Check sheet for the modelled part. Datum: model origin and axes. Units: mm. A direction names the side the tool comes from. Give positions to 0.01 mm unless a question says otherwise; leave off trailing zeros. Order: outer loops, then holes, each group sorted by start corner. A loop starts at its lowest first (then second) coordinate and runs counter-clockwise, first axis right, second up. Notation, with made-up numbers: (18.25, 75) -> (63.25, 75) arc R28 cw to (63.25, 111) -> close; hole circle Ø11 at (42, 76.5). An arc over 180 degrees is marked (long way). Answer in a Markdown table with one row per item. Add a question column.
(1) Go/stop test with flat-tipped pins: pin 1 (24.5 mm diameter, centred on y = -59.5, z = -32, fed in from -X); pin 2 (7 mm diameter, centred on x = -9, z = -56.5, fed in from -Y); pin 3 (12 mm diameter, centred on y = -108.5, z = -31.5, fed in from +X) (3 decimals); pin 4 (5 mm diameter, centred on y = -75.5, z = -14, fed in from -X) (3 decimals). Record where each tip stops, or that it passes through.
(2) Cross-section at A-A (x = 3). Record the cut outline in (y, z) (3 decimals).
(3) Release check for a two-part mould opening along Z. For faces 3 (the face through (10.414, -42, -28)), 4 (the face through (17.145, -96.1, -52.3)), 5 (the face through (-0.263, -75.988, -39.746)) record: released by +Z, released by -Z, zero draft, split by the parting line, or undercut.
(4) Thickness scan on L1, parallel to Z at x = -10, y = -76; L2, parallel to Y at x = 12, z = -20; L3, parallel to Y at x = -11.5, z = -29. Record the ranges inside material, lowest first. Write a range as [from, to].
(5) Set-up check for faces 1 (the face through (-10.414, -42, -28)), 2 (the face through (14.12, -61.63, -33.01)): record each of +Z, -Z, +X, -X, +Y, -Y from which the full face is reachable in a straight line by a thin tool's end or side.
```python
from build123d import *

# Parameters (mm, degrees)
BOSS_EXTRUDE1_DEPTH      = 17.145
BOSS_EXTRUDE1_DEPTH_BACK = 17.145
SKETCH1_R                = 62.865
SKETCH2_R                = 46.355
SKETCH2_R_2              = 33.655
CUT_EXTRUDE1_DEPTH       = 6.731
SKETCH3_R                = 26.289
CUT_EXTRUDE2_DEPTH       = 10.16
BOSS_EXTRUDE2_DEPTH      = 18.796
BOSS_EXTRUDE2_DEPTH_BACK = 18.796
SKETCH4_R                = 14.2875
FILLET1_R                = 6.35
DRAFT1_ANGLE             = 5
DRAFT2_ANGLE             = 5
SKETCH5_R                = 4.826
CUT_EXTRUDE3_DEPTH       = 175.112368419
SKETCH6_W                = 11.857056217
SKETCH6_H                = 6.35
EXTRUDE_THIN1_DEPTH      = 6.35


with BuildPart() as part:
    # Sketch1 → Boss-Extrude1 (new, two sides: drawn at the far end of the back side and taken through both)
    with BuildSketch(Plane(origin=(0, 0, 0), x_dir=(0, 0, -1), z_dir=(1, 0, 0)).offset(-BOSS_EXTRUDE1_DEPTH_BACK)):
        with Locations((34.925, -76.2)):
            Circle(SKETCH1_R)
    extrude(amount=BOSS_EXTRUDE1_DEPTH + BOSS_EXTRUDE1_DEPTH_BACK)

    # Sketch2 → Cut-Extrude1 (cut)
    with BuildSketch(Plane.ZY.offset(17.145)):
        with Locations((-34.925, -76.2)):
            Circle(SKETCH2_R)
        with Locations((-34.925, -76.2)):
            Circle(SKETCH2_R_2, mode=Mode.SUBTRACT)
    cut_extrude1 = extrude(amount=-CUT_EXTRUDE1_DEPTH, mode=Mode.SUBTRACT)

    # Sketch3 → Cut-Extrude2 (cut)
    with BuildSketch(Plane.ZY.offset(17.145)):
        with Locations((-34.925, -76.2)):
            Circle(SKETCH3_R)
    cut_extrude2 = extrude(amount=-CUT_EXTRUDE2_DEPTH, mode=Mode.SUBTRACT)

    # Mirror1: Cut-Extrude1, Cut-Extrude2 across plane
    add(cut_extrude1.mirror(Plane(origin=(0, 0, 0), x_dir=(0, 0, 1), z_dir=(1, 0, 0))), mode=Mode.SUBTRACT)
    add(cut_extrude2.mirror(Plane(origin=(0, 0, 0), x_dir=(0, 0, 1), z_dir=(1, 0, 0))), mode=Mode.SUBTRACT)

    # Sketch4 → Boss-Extrude2 (add, two sides: drawn at the far end of the back side and taken through both)
    with BuildSketch(Plane(origin=(0, 0, 0), x_dir=(0, 0, -1), z_dir=(1, 0, 0)).offset(-BOSS_EXTRUDE2_DEPTH_BACK)):
        with Locations((34.925, -76.2)):
            Circle(SKETCH4_R)
    extrude(amount=BOSS_EXTRUDE2_DEPTH + BOSS_EXTRUDE2_DEPTH_BACK)

    # Fillet1
    fillet1_edges = [part.edges().sort_by_distance(p)[0] for p in [
        (-17.145, -76.2, 27.94),
        (17.145, -76.2, 27.94),
    ]]
    fillet(fillet1_edges, radius=FILLET1_R)

    # Draft1
    draft1_faces = [part.faces().sort_by_distance(p)[0] for p in [
        (-13.7795, -76.2, -81.28),
        (-13.7795, -76.2, -68.58),
        (-12.065, -76.2, -61.214),
        (-12.8905, -76.2, -20.6375),
    ]]
    draft(draft1_faces, Plane(origin=(-18.796, -76.2, -34.925), x_dir=(0, 0, -1), z_dir=(-1, 0, 0)), DRAFT1_ANGLE)

    # Draft2
    draft2_faces = [part.faces().sort_by_distance(p)[0] for p in [
        (13.7795, -76.2, -81.28),
        (13.7795, -76.2, -68.58),
        (12.065, -76.2, -61.214),
        (12.8905, -76.2, -20.6375),
    ]]
    draft(draft2_faces, Plane(origin=(18.796, -76.2, -34.925), x_dir=(0, 0, 1), z_dir=(1, 0, 0)), DRAFT2_ANGLE)

    # Sketch5 → Cut-Extrude3 (cut, through all)
    with BuildSketch(Plane.ZY.offset(18.796)):
        with Locations((-34.925, -76.2)):
            Circle(SKETCH5_R)
    extrude(amount=-CUT_EXTRUDE3_DEPTH, mode=Mode.SUBTRACT)

    # Sketch6 → Extrude-Thin1 (add)
    with BuildSketch(Plane.ZY.offset(6.985)):
        with Locations((-55.141028109, -76.2)):
            Rectangle(SKETCH6_W, SKETCH6_H)
        with Locations((-14.708971892, -76.2)):
            Rectangle(SKETCH6_W, SKETCH6_H)
    extrude(amount=EXTRUDE_THIN1_DEPTH)


solid = part.part
```
Answer below:
| question | item | result |
|---|---|---|
| 1 | pin 1 | stops at x = -18.8 |
| 1 | pin 2 | stops at y = -136.41 |
| 1 | pin 3 | stops at x = 17.145 |
| 1 | pin 4 | stops at x = -13.335 |
| 2 | outline | circle Ø125.73 at (-76.2, -34.925); hole circle Ø9.652 at (-76.2, -34.925) |
| 3 | face 3 | undercut |
| 3 | face 4 | zero draft |
| 3 | face 5 | undercut |
| 4 | L1 | z = [-97.79, -39.75], [-30.1, 27.94] |
| 4 | L2 | y = [-137.15, -119.46], [-107.03, -97.12], [-55.28, -45.37], [-32.94, -15.25] |
| 4 | L3 | y = [-138.75, -121.53], [-109.98, -101.16], [-89.9, -62.5], [-51.24, -42.42], [-30.87, -13.65] |
| 5 | face 1 | -X |
| 5 | face 2 | +X |
